from build123d import *

# Parameters (mm, degrees)
BOSS_EXTRUDE1_DEPTH = 18
CUT_EXTRUDE1_DEPTH  = 214


with BuildPart() as part:
    # Sketch1 → Boss-Extrude1 (new, symmetric)
    with BuildSketch(Plane.XY):
        Polygon((-194, 80), (194, 80), (214, 60), (214, 20), (190, -4), (190, -80), (-190, -80), (-190, -4), (-214, 20), (-214, 60), align=None)
    extrude(amount=BOSS_EXTRUDE1_DEPTH, both=True)

    # Sketch2 → Cut-Extrude1 (cut, symmetric)
    with BuildSketch(Plane(origin=(0, 0, 0), x_dir=(0, 0, -1), z_dir=(1, 0, 0))):
        Polygon((-1, -80), (-18, -59.740188926), (-18, -80), align=None)
        Polygon((1, -80), (18, -59.740188926), (18, -80), align=None)
    extrude(amount=CUT_EXTRUDE1_DEPTH, both=True, mode=Mode.SUBTRACT)


solid = part.part
Can you work these out from the model? Positions are in its coordinate system, mm. A direction names the side the tool comes from. Coordinates: 2 decimals unless noted, no trailing zeros. Write each loop counter-clockwise with the first axis right and the second up, starting at its lowest first coordinate (ties: lowest second). Pieces come first, ordered by that corner, then holes.
Q1. Imagine slicing it at C-C, the plane y = -49. List the corners of the cut face in (x, z) for me, plus the area to 3 significant figures.
Results found:
outline: (-190, -18) - (190, -18) - (190, 18) - (-190, 18) - close
area: 13,700 mm2
Q2. Which directions (+Z, -Z, +X, -X, +Y, -Y) give clear straight access to the entire face, cutting with the end or side of a thin tool? Please do faces 1 (the face through (-190, -34, 0)), 2 (the face through (-2.66, -70.01, 9.38)), 3 (the face through (190, -41, 0)).
Results found:
face 1: +Z, -Z, -X, -Y
face 2: +Z, +X, -X, -Y
face 3: +Z, -Z, +X, -Y
Q3. Imagine slicing it at B-B, the plane z = 8. List the corners of the cut face in (x, y) for me.
Results found:
outline: (-214, 20) - (-190, -4) - (-190, -71.66) - (190, -71.66) - (190, -4) - (214, 20) - (214, 60) - (194, 80) - (-194, 80) - (-214, 60) - close
Q4. Imagine slicing it at A-A, the plane x = -36. List the corners of the cut face in (y, z) for me.
Results found:
outline: (-80, -1) - (-59.74, -18) - (80, -18) - (80, 18) - (-59.74, 18) - (-80, 1) - close
Q5. Please list where these lines run through material, in increasing order: L1, parallel to X at y = -16, z = -2; L2, parallel to Y at x = 145, z = 16.5; L3, parallel to Y at x = 146.5, z = -13.
Results found:
L1: x = -190 to 190
L2: y = -61.53 to 80
L3: y = -65.7 to 80
Q6. For P1, Ø3, axis at x = -106, z = -9, coming from the -Y side; P2, Ø1.5, axis at y = 11, z = -7.5, coming from the -X side; P3, Ø11, axis at y = -54.5, z = 8, coming from the +X side, each with a flat end and sliding along its axis, tell me the tip position at first contact or that it passes through.
Results found:
P1: stops at y = -72.25
P2: stops at x = -205.75
P3: stops at x = 190
